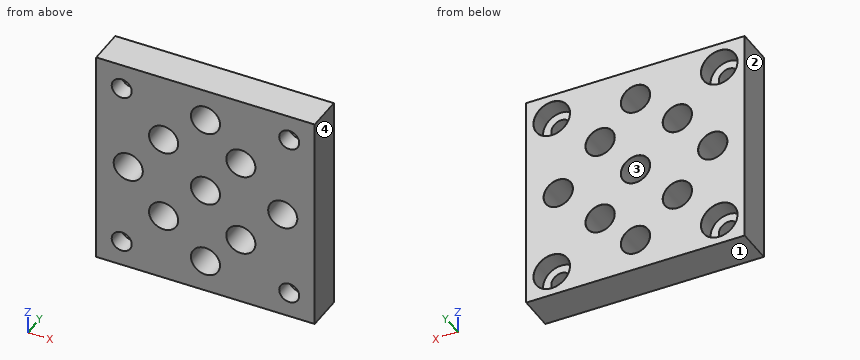
from build123d import *

# Parameters (mm, degrees)
BASE_PLATE_PROFILE_W                   = 60
BASE_PLATE_PROFILE_H                   = 60
BASE_PLATE_60X60X10_DEPTH              = 10
CORNER_COUNTERBORES_M5_SHCS_AT_2_COUNT = 2
CORNER_COUNTERBORES_M5_SHCS_AT_2_PITCH = 46
CORNER_COUNTERBORES_M5_SHCS_AT_3_COUNT = 2
CORNER_COUNTERBORES_M5_SHCS_AT_3_PITCH = 65.053823869
CORNER_COUNTERBORES_M5_SHCS_AT_4_COUNT = 2
CORNER_COUNTERBORES_M5_SHCS_AT_4_PITCH = 46
DOWEL_HOLE_GRID_8_D                    = 8
DOWEL_HOLE_GRID_8_DEPTH                = 35.596557524
DOWEL_HOLE_GRID_8_CSINK_D              = 8.05
DOWEL_HOLE_GRID_8_CSINK_ANGLE          = 100
DOWEL_HOLE_GRID_8_TIP                  = 2.403442476


with BuildPart() as part:
    # Base Plate Profile → Base Plate 60x60x10 (new body)
    with BuildSketch(Plane(origin=(0, 0, 0), x_dir=(1, 0, 0), z_dir=(0, 1, 0))):
        Rectangle(BASE_PLATE_PROFILE_W, BASE_PLATE_PROFILE_H)
    extrude(amount=BASE_PLATE_60X60X10_DEPTH)

    # Sketch3 → Corner Counterbores M5 SHCS (revolve, cut)
    with BuildSketch(Plane(origin=(-23, 10, -23), x_dir=(0, 0, 1), z_dir=(1, 0, 0))):
        Polygon((0, 0), (0, 38), (2.75, 36.347633298), (2.75, 5), (5, 5), (5, 0.020977491), (5.025, 0), align=None)
    corner_counterbores_m5_shcs = revolve(axis=Axis((-23, 16.35, -23), (0, -1, 0)), mode=Mode.SUBTRACT)

    # Corner Counterbores M5 SHCS at 2: Corner Counterbores M5 SHCS ×2
    with Locations(*[(i * CORNER_COUNTERBORES_M5_SHCS_AT_2_PITCH, 0, 0) for i in range(1, CORNER_COUNTERBORES_M5_SHCS_AT_2_COUNT)]):
        add(corner_counterbores_m5_shcs, mode=Mode.SUBTRACT)

    # Corner Counterbores M5 SHCS at 3: Corner Counterbores M5 SHCS ×2
    with Locations(*[Vector(0.7071067811865476, 0, 0.7071067811865476) * (i * CORNER_COUNTERBORES_M5_SHCS_AT_3_PITCH) for i in range(1, CORNER_COUNTERBORES_M5_SHCS_AT_3_COUNT)]):
        add(corner_counterbores_m5_shcs, mode=Mode.SUBTRACT)

    # Corner Counterbores M5 SHCS at 4: Corner Counterbores M5 SHCS ×2
    with Locations(*[(0, 0, i * CORNER_COUNTERBORES_M5_SHCS_AT_4_PITCH) for i in range(1, CORNER_COUNTERBORES_M5_SHCS_AT_4_COUNT)]):
        add(corner_counterbores_m5_shcs, mode=Mode.SUBTRACT)

    # Dowel Hole Grid Ø8
    with Locations(Plane(origin=(0, 10, 0), x_dir=(1, 0, 0), z_dir=(0, 1, 0))):
        with Locations((-21.213203436, 0), (0, 0), (21.213203436, 0), (-11.5, 11.5), (9.713203436, 11.5), (0, 21.213203436), (-11.5, -11.5), (9.713203436, -11.5), (0, -21.213203436)):
            CounterSinkHole(DOWEL_HOLE_GRID_8_D / 2, DOWEL_HOLE_GRID_8_CSINK_D / 2, depth=DOWEL_HOLE_GRID_8_DEPTH, counter_sink_angle=DOWEL_HOLE_GRID_8_CSINK_ANGLE)
            with Locations((0, 0, -(DOWEL_HOLE_GRID_8_DEPTH + DOWEL_HOLE_GRID_8_TIP / 2))):  # 118° drill point
                Cone(0, DOWEL_HOLE_GRID_8_D / 2, DOWEL_HOLE_GRID_8_TIP, mode=Mode.SUBTRACT)


solid = part.part
Build history of the part. All positions in model axes, mm. Face numbers are marked on the shaded views. Give positions to 0.01 mm unless a question says otherwise; leave off trailing zeros. Order: outer loops, then holes, each group sorted by start corner. A loop starts at its lowest first (then second) coordinate and runs counter-clockwise, first axis right, second up. Notation, with made-up numbers: M 62.5,-11 L 84.5,-11 A22 ccw 84.5,9 Z; hole C 86,58 d6. An arc over 180 degrees is marked long. Put each result on its own line as item: value.
Item 1: Slice it at B-B, the plane z = -11.5. Write the cut outline in (x, y) (3 decimals).
From the geometry:
outline: M -30,0 L -15.5,0 L -15.5,9.979 L -15.525,10 L -30,10 Z; M -7.5,0 L 5.713,0 L 5.713,9.979 L 5.688,10 L -7.475,10 L -7.5,9.979 Z; M 13.713,0 L 30,0 L 30,10 L 13.738,10 L 13.713,9.979 Z
Item 2: Two-plate mould, pull along X, no slides. Class the marked faces 1, 2, 3 and 4: +X half, -X half, draft (parallel to the pull), parting line (faces both ways), or undercut.
From the geometry:
face 1: draft
face 2: -X half
face 3: undercut
face 4: +X half
Item 3: Probe line 1 (X direction, y = 2.5, z = 24.5); line 2 (Z direction, x = -23, y = 3.2); line 3 (X direction, y = 8.5, z = -8.5). List the from-to ranges inside material, lowest first. Write a range as [from, to].
From the geometry:
line 1: x = [-30, -25.3], [-20.7, -2.28], [2.28, 20.7], [25.3, 30]
line 2: z = [-30, -25.75], [-20.25, -3.58], [3.58, 20.25], [25.75, 30]
line 3: x = [-30, -14.15], [-8.85, 7.07], [12.36, 30]
Item 4: Slice it at C-C, the plane z = 0. Write the cut outline in (x, y) (3 decimals).
From the geometry:
outline: M -30,0 L -25.213,0 L -25.213,9.979 L -25.238,10 L -30,10 Z; M -17.213,0 L -4,0 L -4,9.979 L -4.025,10 L -17.188,10 L -17.213,9.979 Z; M 4,0 L 17.213,0 L 17.213,9.979 L 17.188,10 L 4.025,10 L 4,9.979 Z; M 25.213,0 L 30,0 L 30,10 L 25.238,10 L 25.213,9.979 Z
Item 5: Slice it at A-A, the plane x = 0. Write the cut outline in (y, z) (3 decimals).
From the geometry:
outline: M 0,-30 L 10,-30 L 10,-25.238 L 9.979,-25.213 L 0,-25.213 Z; M 0,-17.213 L 9.979,-17.213 L 10,-17.188 L 10,-4.025 L 9.979,-4 L 0,-4 Z; M 0,4 L 9.979,4 L 10,4.025 L 10,17.188 L 9.979,17.213 L 0,17.213 Z; M 0,25.213 L 9.979,25.213 L 10,25.238 L 10,30 L 0,30 Z
Item 6: Slice it at D-D, the plane x = -11.5. Write the cut outline in (y, z) (3 decimals).
From the geometry:
outline: M 0,-30 L 10,-30 L 10,-15.525 L 9.979,-15.5 L 0,-15.5 Z; M 0,-7.5 L 9.979,-7.5 L 10,-7.475 L 10,7.475 L 9.979,7.5 L 0,7.5 Z; M 0,15.5 L 9.979,15.5 L 10,15.525 L 10,30 L 0,30 Z
Item 7: Flat gauge pin, fed straight in: pin 1 Ø9 at (x, z) = (-23, 23) entering from +Y. Where does the tip first touch, or does it go through?
From the geometry:
pin 1: stops at y = 5
